Part model, mm, in its own coordinate system. A direction names the side the tool comes from. Round coordinates to 2 decimals unless told otherwise and drop trailing zeros. Write each loop counter-clockwise with the first axis right and the second up, starting at its lowest first coordinate (ties: lowest second). Pieces come first, ordered by that corner, then holes.
from build123d import *

# Parameters (mm, degrees)
BOSS_EXTRUDE1_DEPTH = 300
BOSS_EXTRUDE2_DEPTH = 20
SKETCH3_R           = 20
CUT_EXTRUDE1_DEPTH  = 260


with BuildPart() as part:
    # Sketch1 → Boss-Extrude1 (new body)
    with BuildSketch(Plane(origin=(135.907089576, 362.468590855, 0), x_dir=(0.9363450005078556, -0.35108124419277087, 0), z_dir=(-0.35108124419277087, -0.9363450005078556, 0))):
        with BuildLine():
            ThreePointArc((546.192823225, 2365.719625064), (515.543416647, 2335.070218486), (546.192823225, 2304.420811908))
            ThreePointArc((546.192823225, 2304.420811908), (576.842229803, 2335.070218486), (546.192823225, 2365.719625064))
        make_face()
    extrude(amount=-BOSS_EXTRUDE1_DEPTH)

    # Sketch2 → Boss-Extrude2 (add)
    with BuildSketch(Plane.XY.offset(2344.984494649)):
        with BuildLine():
            Line((750.199941467, 498.038261237), (735.241534602, 458.143707723))
            Line((735.241534602, 458.143707723), (770.071229746, 445.084362397))
            Line((770.071229746, 445.084362397), (785.029636612, 484.978915911))
            ThreePointArc((785.029636612, 484.978915911), (774.144461703, 508.923436146), (750.199941467, 498.038261237))
        make_face()
        with BuildLine():
            ThreePointArc((760.635963738, 485.825631826), (773.297745788, 484.529763272), (774.593614342, 497.191545322))
            ThreePointArc((774.593614342, 497.191545322), (761.931832291, 498.487413876), (760.635963738, 485.825631826))
        make_face(mode=Mode.SUBTRACT)
    extrude(amount=-BOSS_EXTRUDE2_DEPTH)

    # Sketch3 → Cut-Extrude1 (cut)
    with BuildSketch(Plane(origin=(135.907089576, 362.468590855, 0), x_dir=(0.9363450005078556, -0.351081244192771, 0), z_dir=(-0.351081244192771, -0.9363450005078556, 0))):
        with Locations((546.192823225, 2333.834137652)):
            Circle(SKETCH3_R)
    extrude(amount=-CUT_EXTRUDE1_DEPTH, mode=Mode.SUBTRACT)


solid = part.part
Q1. Two-plate mould, pull along Y, no slides. Class faces 1 (the flat face through (777.446, 464.752, 2335.124)), 2 (the flat face through (760, 478, 2344.984)), 3 (the flat face through (742.825, 478.37, 2335.124)): released by +Y, released by -Y, zero draft, split by the parting line, or undercut.
Q2. Drop flat-ended pins along their axis: P1, Ø4, axis at y = 457.5, z = 2358.5, coming from the -X side; P2, Ø2, axis at y = 417.5, z = 2357, coming from the -X side; P3, Ø3, axis at y = 417.5, z = 2339.5, coming from the +X side. Give the stop position or say it passes through.
Q3. Tool access for faces 4 (the flat face through (752.255, 451.765, 2321.877)), 5 (the flat face through (760, 478, 2324.984)), 6 (the flat face through (659.685, 166.079, 2349.121)): list every direction of +Z, -Z, +X, -X, +Y, -Y with a clear straight run to the whole face (end or side of a thin tool).
Q4. Saw through at B-B, the plane y = 468. Write the cut outline in (x, z).
Q5. Saw through at A-A, the plane z = 2359. Write the cut outline in (x, y).
Q6. Wall check: line 1 (Z direction, x = 732, y = 393); line 2 (X direction, y = 250, z = 2325.5); line 3 (X direction, y = 328, z = 2343.5). Give the ranges that are in metal, low to high.
Computed:
1. face 1: undercut
1. face 2: zero draft
1. face 3: released by +Y
2. P1: stops at x = 731.33
2. P2: stops at x = 715.88
2. P3: stops at x = 772.86
3. face 4: none
3. face 5: -Z, +X, +Y
3. face 6: +Z, -Z, -X, -Y
4. outline: (738.94, 2324.98) - (778.66, 2324.98) - (778.66, 2344.98) - (738.94, 2344.98) - close
5. outline: (629.4, 177.43) - (665.26, 163.99) - (770.59, 444.89) - (734.72, 458.34) - close
6. line 1: z = 2304.45 to 2313.87, 2353.8 to 2365.69
6. line 2: x = 645.97 to 657.64, 696.48 to 708.16
6. line 3: x = 674.84 to 687.61, 725.01 to 737.78
